The listing builds one solid part. Answer for the finished solid, in the listing's coordinates (mm). Round coordinates to 2 decimals unless told otherwise and drop trailing zeros. Write each loop counter-clockwise with the first axis right and the second up, starting at its lowest first coordinate (ties: lowest second). Pieces come first, ordered by that corner, then holes. Notation, with made-up numbers: (22, 30.5) - (54, 30.5) arc R21 cw to (54, 54.5) - close; hole circle Ø1 at (60.5, -39.5). An arc over 180 degrees is marked (long way). Return JSON: item names as keys, results as strings. Group by question number.
from build123d import *

# Parameters (mm, degrees)
SKETCH1_R           = 6.25
BOSS_EXTRUDE1_DEPTH = 5


with BuildPart() as part:
    # Sketch1 → Boss-Extrude1 (new body)
    with BuildSketch(Plane.XY.offset(2.5)):
        Polygon((-62, -25), (62, -25), (65, -22), (65, 22), (62, 25), (-62, 25), (-65, 22), (-65, -22), align=None)
        with Locations((-40, 0)):
            Circle(SKETCH1_R, mode=Mode.SUBTRACT)
        with Locations((40, 0)):
            Circle(SKETCH1_R, mode=Mode.SUBTRACT)
    extrude(amount=-BOSS_EXTRUDE1_DEPTH)


solid = part.part
(1) Find section A-A (y = 0). Write down the section's boundary in (x, z), plus the area to 3 significant figures.
(2) Find section C-C (z = 1.55). Write down the section's boundary in (x, y).
(3) Consider line 1 (Y direction, x = -40, z = 1.2); line 2 (X direction, y = 0.5, z = 0.45); line 3 (X direction, y = -4, z = -0.55). Determine where each line is inside the solid, lowest interval first.
(4) Determine the mould class of faces 1 (the cylindrical face through (-34.04, 1.88, 0.04)), 2 (the flat face through (-65, 0, 0)), 3 (the flat face through (-64, -23, 0)) for opening direction Y: +Y half, -Y half, draft (parallel to the pull), parting line (faces both ways), or undercut.
(5) Find section B-B (x = -40). Write down the section's boundary in (y, z).
Check sheet entries:
{
 "1": {"outline": "(-65, -2.5) - (-46.25, -2.5) - (-46.25, 2.5) - (-65, 2.5) - close; (-33.75, -2.5) - (33.75, -2.5) - (33.75, 2.5) - (-33.75, 2.5) - close; (46.25, -2.5) - (65, -2.5) - (65, 2.5) - (46.25, 2.5) - close", "area": "525 mm^2"},
 "2": {"outline": "(-65, -22) - (-62, -25) - (62, -25) - (65, -22) - (65, 22) - (62, 25) - (-62, 25) - (-65, 22) - close; hole circle Ø12.5 at (-40, 0); hole circle Ø12.5 at (40, 0)"},
 "3": {"line 1": "y = -25 to -6.25, 6.25 to 25", "line 2": "x = -65 to -46.23, -33.77 to 33.77, 46.23 to 65", "line 3": "x = -65 to -44.8, -35.2 to 35.2, 44.8 to 65"},
 "4": {"face 1": "undercut", "face 2": "draft", "face 3": "-Y half"},
 "5": {"outline": "(-25, -2.5) - (-6.25, -2.5) - (-6.25, 2.5) - (-25, 2.5) - close; (6.25, -2.5) - (25, -2.5) - (25, 2.5) - (6.25, 2.5) - close"}
}
